```python
from build123d import *

# Parameters (mm, degrees)
SKETCH1_R           = 60
BOSS_EXTRUDE1_DEPTH = 16


with BuildPart() as part:
    # Sketch1 → Boss-Extrude1 (new body)
    with BuildSketch(Plane(origin=(0, 0, 0), x_dir=(1, 0, 0), z_dir=(0, 1, 0))):
        with BuildLine():
            Line((-124.5, 0), (124.5, 0))
            Line((124.5, 0), (136.5, 12))
            Line((136.5, 12), (136.5, 160.6))
            ThreePointArc((136.5, 160.6), (131.600675284, 175.464819311), (118.822971749, 184.503432489))
            Line((118.822971749, 184.503432489), (10.252160448, 217.764805485))
            ThreePointArc((10.252160448, 217.764805485), (0, 219.3), (-10.252160448, 217.764805485))
            Line((-10.252160448, 217.764805485), (-118.822971749, 184.503432489))
            ThreePointArc((-118.822971749, 184.503432489), (-131.600675284, 175.464819311), (-136.5, 160.6))
            Line((-136.5, 160.6), (-136.5, 12))
            Line((-136.5, 12), (-124.5, 0))
        make_face()
        with Locations(Location((0, 96, 0), (0, 0, 270))):
            Circle(SKETCH1_R, mode=Mode.SUBTRACT)
    extrude(amount=BOSS_EXTRUDE1_DEPTH)


solid = part.part
```
Can you work these out from the model? Positions are in its coordinate system, mm. Give positions to 0.01 mm unless a question says otherwise; leave off trailing zeros. Loops run counter-clockwise (first coordinate to the right, second up) from the corner with the lowest first, then second, coordinate; pieces in that order, holes last. Notation, with made-up numbers: M 46.5,71.5 L 76.5,71.5 A17 ccw 76.5,89.5 Z; hole C -7.5,49 d10. An arc over 180 degrees is marked long. One line per item, written item: value.
(1) Suppose I cut it at A-A on z = -96. List the corners of the cut face in (x, y) for me.
Returned:
outline: M -136.5,0 L -60,0 L -60,16 L -136.5,16 Z; M 60,0 L 136.5,0 L 136.5,16 L 60,16 Z
(2) We'd pull the mould along X, two halves only. Please class faces 1 (the face through (-63.778, 7.888, -201.367)), 2 (the face through (-2, 16, -160)), 3 (the face through (0.1, 7.9, -219.3)), 4 (the face through (2.64, 7.89, -155.94)): released by +X, released by -X, zero draft, split by the parting line, or undercut.
Returned:
face 1: released by -X
face 2: zero draft
face 3: split by the parting line
face 4: undercut
(3) Will this pin go through, and if not, where does the flat tip stop? pin 1 (8 mm diameter, centred on x = -57.5, y = 13.5, fed in from -Z).
Returned:
pin 1: z = -204.52
(4) I need wall thicknesses on line 1 (X direction, y = 7.5, z = -96); line 2 (X direction, y = 6.75, z = -93.5); line 3 (Z direction, x = -27.5, y = 7.25). Which ranges of each line are inside material? Lowest first, please.
Returned:
line 1: -136.5 to -60, 60 to 136.5
line 2: -136.5 to -59.95, 59.95 to 136.5
line 3: -212.48 to -149.33, -42.67 to 0
(5) Suppose I cut it at C-C on y = 5. List the corners of the cut face in (x, z) for me, plus the area to 3 significant figures.
Returned:
outline: M -136.5,-160.6 A25 ccw -118.82,-184.5 L -10.25,-217.76 A35 ccw 10.25,-217.76 L 118.82,-184.5 A25 ccw 136.5,-160.6 L 136.5,-12 L 124.5,0 L -124.5,0 L -136.5,-12 Z; hole C 0,-96 d120
area: 43,000 mm^2
(6) Suppose I cut it at D-D on z = -175.5. List the corners of the cut face in (x, y) for me, plus the area to 3 significant figures.
Returned:
outline: M -131.57,0 L 131.57,0 L 131.57,16 L -131.57,16 Z
area: 4,210 mm^2
(7) Suppose I cut it at B-B on x = 0. List the corners of the cut face in (y, z) for me.
Returned:
outline: M 0,-219.3 L 16,-219.3 L 16,-156 L 0,-156 Z; M 0,-36 L 16,-36 L 16,0 L 0,0 Z
